Build history of the part. All positions in model axes, mm. Round coordinates to 2 decimals unless told otherwise and drop trailing zeros. Write each loop counter-clockwise with the first axis right and the second up, starting at its lowest first coordinate (ties: lowest second). Pieces come first, ordered by that corner, then holes. Notation, with made-up numbers: (30, 66) - (84, 66) arc R14 ccw to (84, 78) - close; hole circle Ø11 at (-35, -32). An arc over 180 degrees is marked (long way). One line per question, with ' | ' between items.
from build123d import *

# Parameters (mm, degrees)
SKETCH1_W            = 360
SKETCH1_H            = 360
EXTRUDE1_DEPTH       = 10
M24_TAPPED_HOLE1_D   = 21
LPATTERN2_COUNT      = 2
LPATTERN2_PITCH      = 144
LPATTERN2_COUNT_DIR2 = 2
LPATTERN2_PITCH_DIR2 = 266


with BuildPart() as part:
    # Sketch1 → Extrude1 (new, symmetric)
    with BuildSketch(Plane(origin=(0, 0, 0), x_dir=(1, 0, 0), z_dir=(0, 1, 0))):
        Rectangle(SKETCH1_W, SKETCH1_H)
    extrude(amount=EXTRUDE1_DEPTH, both=True)

    # M24 Tapped Hole1 (through all)
    with Locations(Plane(origin=(0, 10, 0), x_dir=(-1, 0, 0), z_dir=(0, 1, 0))):
        with Locations((133, -72)):
            m24_tapped_hole1 = Hole(M24_TAPPED_HOLE1_D / 2)

    # LPattern2: M24 Tapped Hole1 2 × 2
    with Locations(*[(j * LPATTERN2_PITCH_DIR2, 0, i * LPATTERN2_PITCH) for i in range(LPATTERN2_COUNT) for j in range(LPATTERN2_COUNT_DIR2) if (i, j) != (0, 0)]):
        add(m24_tapped_hole1, mode=Mode.SUBTRACT)


solid = part.part
Q1. Pull direction Z, two halves, no side cores. Call faces 1 (the flat face through (-3, 0, -180)), 2 (the flat face through (-3, 0, 180)), 3 (the cylindrical face through (-140.739, -0.14, 79.096)), 4 (the flat face through (-3, 10, -3)): +Z half, -Z half, draft (parallel to the pull), parting line (faces both ways), or undercut.
Found:
face 1: -Z half | face 2: +Z half | face 3: undercut | face 4: draft
Q2. Drill centre lines: L1, parallel to Z at x = -133, y = 3.75; L2, parallel to Z at x = -140, y = -5. Where is each one in solid material? Low to high. Write a range as from..to.
Found:
L1: -180..-82.5, -61.5..61.5, 82.5..180 | L2: -180..-79.83, -64.17..64.17, 79.83..180
Q3. Saw through at B-B, the plane x = -133. List the corners of the cut face in (y, z).
Found:
outline: (-10, -180) - (10, -180) - (10, -82.5) - (-10, -82.5) - close; (-10, -61.5) - (10, -61.5) - (10, 61.5) - (-10, 61.5) - close; (-10, 82.5) - (10, 82.5) - (10, 180) - (-10, 180) - close
Q4. Saw through at A-A, the plane z = 72. List the corners of the cut face in (x, y).
Found:
outline: (-180, -10) - (-143.5, -10) - (-143.5, 10) - (-180, 10) - close; (-122.5, -10) - (122.5, -10) - (122.5, 10) - (-122.5, 10) - close; (143.5, -10) - (180, -10) - (180, 10) - (143.5, 10) - close
